Read the model definition and answer for the solid it produces. Units are mm, in the model's axes. A direction names the side the tool comes from. Coordinates: 2 decimals unless noted, no trailing zeros. Order: outer loops, then holes, each group sorted by start corner. A loop starts at its lowest first (then second) coordinate and runs counter-clockwise, first axis right, second up. Notation, with made-up numbers: M 12.25,34 L 56.25,34 A17 ccw 56.25,63 Z; hole C 56,-32.75 d4. An arc over 180 degrees is marked long. Put each result on its own line as item: value.
from build123d import *

# Parameters (mm, degrees)
SKETCH_1_W      = 2
SKETCH_1_H      = 28
SKETCH_1_W_2    = 12
SKETCH_1_H_2    = 7
SKETCH_1_R      = 1.55
EXTRUDE_1_DEPTH = 4.8
FILLET_1_R      = 1


with BuildPart() as part:
    # 草图1 → 凸台-拉伸1 (new body)
    # profile 1 of 4: a face of its own
    with BuildSketch(Plane(origin=(0, 0, 0), x_dir=(1, 0, 0), z_dir=(0, 1, 0))):
        with Locations((-5, 17.5)):
            Rectangle(SKETCH_1_W, SKETCH_1_H)
    # profile 2 of 4: a face of its own
    with BuildSketch(Plane(origin=(0, 0, 0), x_dir=(1, 0, 0), z_dir=(0, 1, 0))):
        with Locations((0, 35)):
            Rectangle(SKETCH_1_W_2, SKETCH_1_H_2)
        with Locations(Location((0, 35, 0), (0, 0, 270))):
            Circle(SKETCH_1_R, mode=Mode.SUBTRACT)
    # profile 3 of 4: a face of its own
    with BuildSketch(Plane(origin=(0, 0, 0), x_dir=(1, 0, 0), z_dir=(0, 1, 0))):
        with Locations((5, 17.5)):
            Rectangle(SKETCH_1_W, SKETCH_1_H)
    # profile 4 of 4: a face of its own
    with BuildSketch(Plane(origin=(0, 0, 0), x_dir=(1, 0, 0), z_dir=(0, 1, 0))):
        Rectangle(SKETCH_1_W_2, SKETCH_1_H_2)
        with Locations(Location((0, 0, 0), (0, 0, 270))):
            Circle(SKETCH_1_R, mode=Mode.SUBTRACT)
    extrude(amount=EXTRUDE_1_DEPTH)

    # 圆角1
    fillet_1_edges = [part.edges().sort_by_distance(p)[0] for p in [
        (-4, 2.4, -3.5),
        (4, 2.4, -3.5),
        (4, 2.4, -31.5),
        (-4, 2.4, -31.5),
        (6, 2.4, 3.5),
        (-6, 2.4, 3.5),
        (-6, 2.4, -38.5),
        (6, 2.4, -38.5),
    ]]
    fillet(fillet_1_edges, radius=FILLET_1_R)


solid = part.part
Q1. Given pin 1 (1 mm diameter, centred on x = -2, z = -22, fed in from +Y), flat-ended and moving along its own axis, determine where the tip first touches the part or whether it passes through.
Answers below:
pin 1: passes through
Q2. Find section C-C on x = -2.25. Write down the section's boundary in (y, z), plus the area to 3 significant figures.
Answers below:
outline: M 0,-38.5 L 4.8,-38.5 L 4.8,-31.5 L 0,-31.5 Z; M 0,-3.5 L 4.8,-3.5 L 4.8,3.5 L 0,3.5 Z
area: 67.2 mm^2
Q3. A tool of negligible diameter and unlimited length cuts with its end or side. For faces 4 (the face through (4, 2, -17)), 5 (the face through (-6, 2, -17)), from which of +Z, -Z, +X, -X, +Y, -Y can it reach the whole face along a straight path? Write none if from no direction.
Answers below:
face 4: +Y, -Y
face 5: +Z, -Z, -X, +Y, -Y
Q4. Find section D-D on x = 0. Write down the section's boundary in (y, z).
Answers below:
outline: M 0,-38.5 L 4.8,-38.5 L 4.8,-36.55 L 0,-36.55 Z; M 0,-33.45 L 4.8,-33.45 L 4.8,-31.5 L 0,-31.5 Z; M 0,-3.5 L 4.8,-3.5 L 4.8,-1.55 L 0,-1.55 Z; M 0,1.55 L 4.8,1.55 L 4.8,3.5 L 0,3.5 Z
Q5. For a pull along X with two mould halves and no side action, classify faces 1 (the face through (-5, 4.8, -18)), 2 (the face through (5.715, 2.434, 3.199)), 3 (the face through (3.715, 2.434, -31.199)) as +X half, -X half, draft (parallel to the pull), parting line (faces both ways), or undercut.
Answers below:
face 1: draft
face 2: +X half
face 3: undercut
Q6. Find section A-A on z = 0. Write down the section's boundary in (x, y).
Answers below:
outline: M -6,0 L -1.55,0 L -1.55,4.8 L -6,4.8 Z; M 1.55,0 L 6,0 L 6,4.8 L 1.55,4.8 Z
Q7. Consider line 1 along X through (y, z) = (2.3, 0); line 2 along X through (y, z) = (2.1, -6); line 3 along Z through (x, y) = (3, 4.4). Determine where each line is inside the solid, lowest interval first.
Answers below:
line 1: x = -6 to -1.55, 1.55 to 6
line 2: x = -6 to -4, 4 to 6
line 3: z = -38.5 to -31.5, -3.5 to 3.5
Q8. Find section B-B on y = 3.7. Write down the section's boundary in (x, z), plus the area to 3 significant figures.
Answers below:
outline: M -6,-37.5 A1 ccw -5,-38.5 L 5,-38.5 A1 ccw 6,-37.5 L 6,2.5 A1 ccw 5,3.5 L -5,3.5 A1 ccw -6,2.5 Z; hole M -4,-30.5 A1 ccw -3,-31.5 L 3,-31.5 A1 ccw 4,-30.5 L 4,-4.5 A1 ccw 3,-3.5 L -3,-3.5 A1 ccw -4,-4.5 Z; hole C 0,-35 d3.1; hole C 0,0 d3.1
area: 265 mm^2
